```python
from build123d import *

# Parameters (mm, degrees)
EXTRUDE_1_DEPTH     = 95
SKETCH_2_R          = 2.75
CUT_EXTRUDE_1_DEPTH = 113.405897954
SKETCH_3_R          = 5
CUT_EXTRUDE_2_DEPTH = 5.75
SKETCH_4_W          = 12
SKETCH_4_H          = 24
CUT_EXTRUDE_3_DEPTH = 124.632519994
SKETCH_5_R          = 1.25
CUT_EXTRUDE_4_DEPTH = 7.5
SKETCH_6_R          = 1.5
CUT_EXTRUDE_5_DEPTH = 6
SKETCH_7_R          = 8
CUT_EXTRUDE_6_DEPTH = 124.632519994


with BuildPart() as part:
    # 草图1 → 凸台-拉伸1 (new body)
    with BuildSketch(Plane.XY):
        Polygon((-42.966101695, 24), (-42.966101695, -28), (31.033898305, -28), (31.033898305, 24), (23.033898305, 24), (23.033898305, 0), (18.033898305, 0), (18.033898305, -18), (-29.966101695, -18), (-29.966101695, 0), (-34.966101695, 0), (-34.966101695, 24), align=None)
    extrude(amount=EXTRUDE_1_DEPTH)

    # 草图2 → 切除-拉伸1 (cut, through all)
    with BuildSketch(Plane(origin=(0, -18, 0), x_dir=(1, 0, 0), z_dir=(0, 1, 0))):
        with Locations(Location((-19.966101695, -10, 0), (0, 0, 270))):
            Circle(SKETCH_2_R)
        with Locations(Location((-19.966101695, -50, 0), (0, 0, 270))):
            Circle(SKETCH_2_R)
        with Locations(Location((8.033898305, -10, 0), (0, 0, 270))):
            Circle(SKETCH_2_R)
        with Locations(Location((8.033898305, -50, 0), (0, 0, 270))):
            Circle(SKETCH_2_R)
    extrude(amount=-CUT_EXTRUDE_1_DEPTH, mode=Mode.SUBTRACT)

    # 草图3 → 切除-拉伸2 (cut)
    with BuildSketch(Plane(origin=(0, -18, 0), x_dir=(1, 0, 0), z_dir=(0, 1, 0))):
        with Locations(Location((-19.966101695, -10, 0), (0, 0, 270))):
            Circle(SKETCH_3_R)
        with Locations(Location((-19.966101695, -50, 0), (0, 0, 270))):
            Circle(SKETCH_3_R)
        with Locations(Location((8.033898305, -10, 0), (0, 0, 270))):
            Circle(SKETCH_3_R)
        with Locations(Location((8.033898305, -50, 0), (0, 0, 270))):
            Circle(SKETCH_3_R)
    extrude(amount=-CUT_EXTRUDE_2_DEPTH, mode=Mode.SUBTRACT)

    # 草图4 → 切除-拉伸3 (cut, through all)
    with BuildSketch(Plane.ZY.offset(42.966101695)):
        with Locations((6, 12)):
            Rectangle(SKETCH_4_W, SKETCH_4_H)
    extrude(amount=-CUT_EXTRUDE_3_DEPTH, mode=Mode.SUBTRACT)

    # 草图5 → 切除-拉伸4 (cut)
    with BuildSketch(Plane(origin=(0, 0, 0), x_dir=(1, 0, 0), z_dir=(0, 1, 0))):
        with Locations(Location((-32.466101695, -10, 0), (0, 0, 270))):
            Circle(SKETCH_5_R)
        with Locations(Location((20.533898305, -10, 0), (0, 0, 270))):
            Circle(SKETCH_5_R)
    extrude(amount=-CUT_EXTRUDE_4_DEPTH, mode=Mode.SUBTRACT)

    # 草图6 → 切除-拉伸5 (cut)
    with BuildSketch(Plane(origin=(0, 0, 0), x_dir=(1, 0, 0), z_dir=(0, 1, 0))):
        with Locations(Location((-32.466101695, -10, 0), (0, 0, 270))):
            Circle(SKETCH_6_R)
        with Locations(Location((20.533898305, -10, 0), (0, 0, 270))):
            Circle(SKETCH_6_R)
    extrude(amount=-CUT_EXTRUDE_5_DEPTH, mode=Mode.SUBTRACT)

    # 草图7 → 切除-拉伸6 (cut, through all)
    with BuildSketch(Plane.ZY.offset(42.966101695)):
        with Locations((30, 10)):
            Circle(SKETCH_7_R)
    extrude(amount=-CUT_EXTRUDE_6_DEPTH, mode=Mode.SUBTRACT)


solid = part.part
```
Model file for the job. Use its own axes, mm. A direction names the side the tool comes from. Round coordinates to 2 decimals unless told otherwise and drop trailing zeros. Write each loop counter-clockwise with the first axis right and the second up, starting at its lowest first coordinate (ties: lowest second). Pieces come first, ordered by that corner, then holes. Notation, with made-up numbers: (63.5, 16) -> (100.5, 16) arc R16 ccw to (100.5, 33) -> close; hole circle Ø1 at (51.25, -11.5). An arc over 180 degrees is marked (long way). Answer as CSV lines item,"result".
1. Slice it at B-B, the plane z = 30. List the corners of the cut face in (x, y).
Resolved:
outline,"(-42.97, -28) -> (31.03, -28) -> (31.03, 2) -> (23.03, 2) -> (23.03, 0) -> (18.03, 0) -> (18.03, -18) -> (-29.97, -18) -> (-29.97, 0) -> (-34.97, 0) -> (-34.97, 2) -> (-42.97, 2) -> close; (-42.97, 18) -> (-34.97, 18) -> (-34.97, 24) -> (-42.97, 24) -> close; (23.03, 18) -> (31.03, 18) -> (31.03, 24) -> (23.03, 24) -> close"
2. Slice it at C-C, the plane y = 10. List the corners of the cut face in (x, z).
Resolved:
outline,"(-42.97, 12) -> (-34.97, 12) -> (-34.97, 22) -> (-42.97, 22) -> close; (-42.97, 38) -> (-34.97, 38) -> (-34.97, 95) -> (-42.97, 95) -> close; (23.03, 12) -> (31.03, 12) -> (31.03, 22) -> (23.03, 22) -> close; (23.03, 38) -> (31.03, 38) -> (31.03, 95) -> (23.03, 95) -> close"
3. Pin check, flat tips, straight feed: pin 1 Ø4 at (x, z) = (-4.5, 44.5) entering from +Y; pin 2 Ø3 at (x, z) = (-32, 9.5) entering from +Y; pin 3 Ø6.5 at (x, y) = (27.5, 16) entering from -Z. Stop position of each tip, or through.
Resolved:
pin 1,"y = -18"
pin 2,"y = 0"
pin 3,"z = 12"
4. Mould opens along Z. For faces 4 (the face through (-42.966, -2, 47)), 5 (the face through (-39, 12, 12)), 6 (the face through (-20, -21, 45)) say: +Z half, -Z half, draft (parallel to the pull), parting line (faces both ways), or undercut.
Resolved:
face 4,"draft"
face 5,"-Z half"
face 6,"undercut"
5. Drill centre lines: line 1 (X direction, y = -6.75, z = 10); line 2 (X direction, y = -20.7, z = 10); line 3 (X direction, y = -25.9, z = 50). Where is each one in solid material? Low to high.
Resolved:
line 1,"-42.97 to -33.72, -31.22 to -29.97, 18.03 to 19.28, 21.78 to 31.03"
line 2,"-42.97 to -24.97, -14.97 to 3.03, 13.03 to 31.03"
line 3,"-42.97 to -22.72, -17.22 to 5.28, 10.78 to 31.03"
6. Slice it at A-A, the plane y = -12. List the corners of the cut face in (x, z).
Resolved:
outline,"(-42.97, 0) -> (-29.97, 0) -> (-29.97, 95) -> (-42.97, 95) -> close; (18.03, 0) -> (31.03, 0) -> (31.03, 95) -> (18.03, 95) -> close"
7. Slice it at D-D, the plane z = 79.5. List the corners of the cut face in (x, y).
Resolved:
outline,"(-42.97, -28) -> (31.03, -28) -> (31.03, 24) -> (23.03, 24) -> (23.03, 0) -> (18.03, 0) -> (18.03, -18) -> (-29.97, -18) -> (-29.97, 0) -> (-34.97, 0) -> (-34.97, 24) -> (-42.97, 24) -> close"
8. Tool access for faces 1 (the face through (-33.93, -2.96, 9.67)), 2 (the face through (-34.966, 12, 53)), 3 (the face through (27, 10, 22)): list every direction of +Z, -Z, +X, -X, +Y, -Y with a clear straight run to the whole face (end or side of a thin tool).
Resolved:
face 1,"+Y"
face 2,"+Z, -Z, +Y"
face 3,"+X, -X"
